Check sheet for the modelled part. Datum: model origin and axes. Units: mm. Face numbers are marked on the shaded views. A direction names the side the tool comes from. Give positions to 0.01 mm unless a question says otherwise; leave off trailing zeros. Order: outer loops, then holes, each group sorted by start corner. A loop starts at its lowest first (then second) coordinate and runs counter-clockwise, first axis right, second up. Notation, with made-up numbers: (0, 60) - (18, 60) arc R31 cw to (18, 96) - close; hole circle Ø11 at (-34.5, -38.5). An arc over 180 degrees is marked (long way). Answer in a Markdown table with one row per item.
from build123d import *

# Parameters (mm, degrees)
BOSS_EXTRUDE1_DEPTH = 7.5
SKETCH2_R           = 3.4
CUT_EXTRUDE1_DEPTH  = 15
SKETCH4_R           = 19
CUT_EXTRUDE3_DEPTH  = 84.988094394
SKETCH3_R           = 21
CUT_EXTRUDE4_DEPTH  = 12
M4_TAPPED_HOLE2_D   = 3.3
M4_TAPPED_HOLE1_D   = 3.3
FILLET2_R           = 5


with BuildPart() as part:
    # Sketch1 → Boss-Extrude1 (new, symmetric)
    with BuildSketch(Plane.XY):
        Polygon((30, 0), (-30, 0), (-30, 10), (-15, 10), (-15, 25), (-30, 25), (-30, 77), (30, 77), (30, 25), (15, 25), (15, 10), (30, 10), align=None)
    extrude(amount=BOSS_EXTRUDE1_DEPTH, both=True)

    # Sketch2 → Cut-Extrude1 (cut)
    with BuildSketch(Plane.XZ):
        with Locations(Location((-25, 0, 0), (0, 0, 270))):
            Circle(SKETCH2_R)
        with Locations(Location((25, 0, 0), (0, 0, 270))):
            Circle(SKETCH2_R)
    extrude(amount=-CUT_EXTRUDE1_DEPTH, mode=Mode.SUBTRACT)

    # Sketch4 → Cut-Extrude3 (cut, through all)
    with BuildSketch(Plane.XY.offset(7.5)):
        with Locations((0, 52)):
            Circle(SKETCH4_R)
    extrude(amount=-CUT_EXTRUDE3_DEPTH, mode=Mode.SUBTRACT)

    # Sketch3 → Cut-Extrude4 (cut)
    with BuildSketch(Plane.XY.offset(7.5)):
        with Locations((0, 52)):
            Circle(SKETCH3_R)
    extrude(amount=-CUT_EXTRUDE4_DEPTH, mode=Mode.SUBTRACT)

    # M4 Tapped Hole2 (through all)
    with Locations(Plane.XY.offset(7.5)):
        with Locations((24, 52), (-24, 52)):
            Hole(M4_TAPPED_HOLE2_D / 2)

    # M4 Tapped Hole1 (through all)
    with Locations(Plane.XY.offset(7.5)):
        with Locations((-25, 72), (25, 72)):
            Hole(M4_TAPPED_HOLE1_D / 2)

    # Fillet2
    fillet2_edges = [part.edges().sort_by_distance(p)[0] for p in [
        (-30, 25, 0),
        (-30, 77, 0),
        (30, 77, 0),
        (30, 25, 0),
        (15, 25, 0),
        (15, 10, 0),
        (-15, 10, 0),
        (-15, 25, 0),
    ]]
    fillet(fillet2_edges, radius=FILLET2_R)


solid = part.part
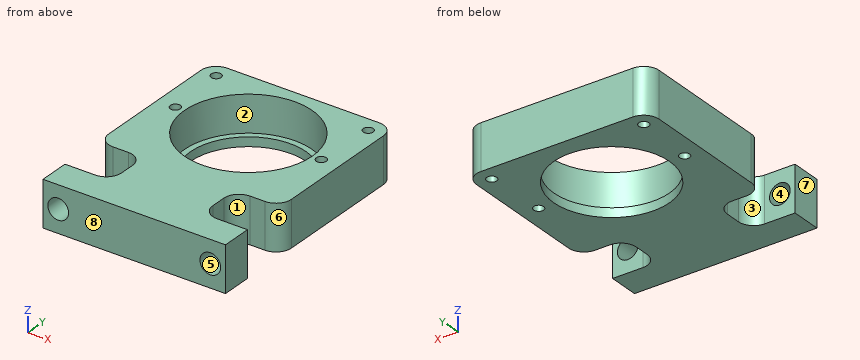
(1) Gauge pin test, flat ends, axial feed: P1, Ø4, axis at y = 17, z = -1.5, coming from the +X side; P2, Ø2.5, axis at y = 17.5, z = 2.5, coming from the -X side; P3, Ø6, axis at x = -25, z = 0, coming from the -Y side. Record the tip position at first contact, or that the pin passes through.
Geometry says:
| item | result |
|---|---|
| P1 | x = 15 |
| P2 | x = -15 |
| P3 | y = 25 |
(2) Cross-section at B-B, the plane x = 0. Record the cut outline in (y, z), then the cut area to 3 significant figures.
Geometry says:
| item | result |
|---|---|
| outline | (0, -7.5) - (33, -7.5) - (33, -4.5) - (31, -4.5) - (31, 7.5) - (0, 7.5) - close; (71, -7.5) - (77, -7.5) - (77, 7.5) - (73, 7.5) - (73, -4.5) - (71, -4.5) - close |
| area | 537 mm² |
(3) Cross-section at D-D, the plane x = 17. Record the cut outline in (y, z), then the cut area to 3 significant figures.
Geometry says:
| item | result |
|---|---|
| outline | (0, -7.5) - (11, -7.5) - (11, 7.5) - (0, 7.5) - close; (24, -7.5) - (43.51, -7.5) - (43.51, -4.5) - (39.67, -4.5) - (39.67, 7.5) - (24, 7.5) - close; (60.49, -7.5) - (77, -7.5) - (77, 7.5) - (64.33, 7.5) - (64.33, -4.5) - (60.49, -4.5) - close |
| area | 613 mm² |
(4) Cross-section at C-C, the plane y = 48. Record the cut outline in (x, z).
Geometry says:
| item | result |
|---|---|
| outline | (-30, -7.5) - (-18.57, -7.5) - (-18.57, -4.5) - (-20.62, -4.5) - (-20.62, 7.5) - (-30, 7.5) - close; (18.57, -7.5) - (30, -7.5) - (30, 7.5) - (20.62, 7.5) - (20.62, -4.5) - (18.57, -4.5) - close |
(5) Thickness scan on L1, parallel to Y at x = 16.5, z = -5; L2, parallel to X at y = 2.75, z = 0; L3, parallel to Y at x = 24, z = 1. Record the ranges inside material, lowest first.
Geometry says:
| item | result |
|---|---|
| L1 | 0 to 11.43, 23.57 to 42.58, 61.42 to 77 |
| L2 | -30 to -28.4, -21.6 to 21.6, 28.4 to 30 |
| L3 | 25 to 50.35, 53.65 to 70.69, 73.31 to 77 |
(6) Access from +Z, -Z, +X, -X, +Y, -Y to the whole of each face (thin tool, end or side, straight path). Record for the marked faces 1, 2, 3 and 4.
Geometry says:
| item | result |
|---|---|
| face 1 | +Z, -Z, +X |
| face 2 | +Z |
| face 3 | +Z, -Z, -X |
| face 4 | -Y |
(7) Cross-section at A-A, the plane z = 1.75. Give the number of separate pieces and of enclosed holes in the cut face, then the cut area to 3 significant figures.
Geometry says:
| item | result |
|---|---|
| separate pieces | 3 |
| enclosed holes | 5 |
| area | 2,630 mm² |
(8) Mould release check, pull along X, two halves, no side actions. Record for the marked faces 5, 6, 7 and 8: pulls with the +X half, pulls with the -X half, needs draft (parallel to the pull), parting line crosses it, or undercut.
Geometry says:
| item | result |
|---|---|
| face 5 | undercut |
| face 6 | pulls with the +X half |
| face 7 | pulls with the -X half |
| face 8 | needs draft |
